Input: part model. Units: mm. Frame: model coordinates. Give positions to 0.01 mm unless a question says otherwise; leave off trailing zeros. Loops run counter-clockwise (first coordinate to the right, second up) from the corner with the lowest first, then second, coordinate; pieces in that order, holes last.
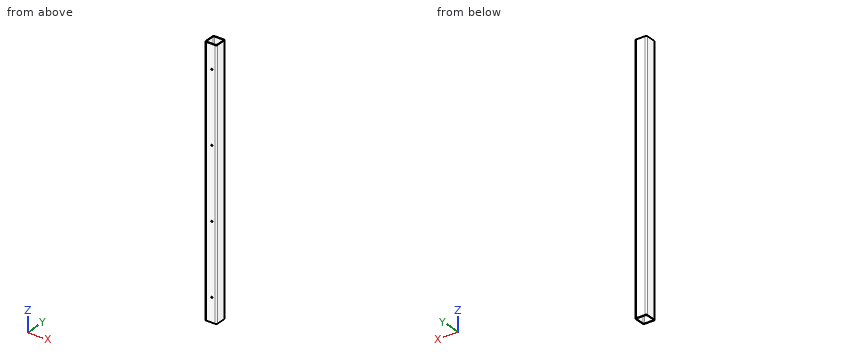
from build123d import *

# Parameters (mm, degrees)
GB_6728_1986_050_X_50_X_3_1_DEPTH = 1100
HOLE_WIZARD_M6_1_D                = 5
HOLE_WIZARD_M6_1_DEPTH            = 15
HOLE_WIZARD_M6_1_TIP              = 1.502151548


with BuildPart() as part:
    # Sketch1 → Gb／6728-1986方形空心型钢 050 X 50 X 3(1) (new body)
    with BuildSketch(Plane(origin=(0, 0, 0), x_dir=(-1, 0, 0), z_dir=(0, 0, -1))):
        with BuildLine():
            Line((-19, -25), (19, -25))
            ThreePointArc((19, -25), (23.242640687, -23.242640687), (25, -19))
            Line((25, -19), (25, 19))
            ThreePointArc((25, 19), (23.242640687, 23.242640687), (19, 25))
            Line((19, 25), (-19, 25))
            ThreePointArc((-19, 25), (-23.242640687, 23.242640687), (-25, 19))
            Line((-25, 19), (-25, -19))
            ThreePointArc((-25, -19), (-23.242640687, -23.242640687), (-19, -25))
        make_face()
        with BuildLine():
            Line((-19, -22), (19, -22))
            ThreePointArc((19, -22), (21.121320344, -21.121320344), (22, -19))
            Line((22, -19), (22, 19))
            ThreePointArc((22, 19), (21.121320344, 21.121320344), (19, 22))
            Line((19, 22), (-19, 22))
            ThreePointArc((-19, 22), (-21.121320344, 21.121320344), (-22, 19))
            Line((-22, 19), (-22, -19))
            ThreePointArc((-22, -19), (-21.121320344, -21.121320344), (-19, -22))
        make_face(mode=Mode.SUBTRACT)
    extrude(amount=GB_6728_1986_050_X_50_X_3_1_DEPTH)

    # M6 螺纹孔1
    with Locations(Plane(origin=(0, -25, 0), x_dir=(-1, 0, 0), z_dir=(0, -1, 0))):
        with Locations((-5, 100), (-5, 400), (-5, 700), (-5, 1000)):
            Hole(HOLE_WIZARD_M6_1_D / 2, depth=HOLE_WIZARD_M6_1_DEPTH)
            with Locations((0, 0, -(HOLE_WIZARD_M6_1_DEPTH + HOLE_WIZARD_M6_1_TIP / 2))):  # 118° drill point
                Cone(0, HOLE_WIZARD_M6_1_D / 2, HOLE_WIZARD_M6_1_TIP, mode=Mode.SUBTRACT)


solid = part.part
(1) Ray query, probe 1 along Z at (x, y) = (5, -23.35); probe 2 along Y at (x, z) = (17.5, -656.5). Return the intervals inside material, ascending.
Values follow:
probe 1: z = -1100 to -1002.5, -997.5 to -702.5, -697.5 to -402.5, -397.5 to -102.5, -97.5 to 0
probe 2: y = -25 to -22, 22 to 25
(2) Cut plane A-A (x = -6.5). Return the cut outline in (y, z).
Values follow:
outline: (-25, -1100) - (-22, -1100) - (-22, 0) - (-25, 0) - close; (22, -1100) - (25, -1100) - (25, 0) - (22, 0) - close
(3) Cut plane C-C (z = -234). Return the cut outline in (x, y), and give its area (3 significant figures).
Values follow:
outline: (-25, -19) arc R6 ccw to (-19, -25) - (19, -25) arc R6 ccw to (25, -19) - (25, 19) arc R6 ccw to (19, 25) - (-19, 25) arc R6 ccw to (-25, 19) - close; hole (-22, -19) arc R3 ccw to (-19, -22) - (19, -22) arc R3 ccw to (22, -19) - (22, 19) arc R3 ccw to (19, 22) - (-19, 22) arc R3 ccw to (-22, 19) - close
area: 541 mm2
(4) Pin query (flat end, axial travel): pin 1 Ø3 at (x, z) = (5, -700) entering from -Y. Return the tip coordinate at first contact, or that it passes through.
Values follow:
pin 1: stops at y = 22
